```python
from build123d import *

# Parameters (mm, degrees)
SKETCH_1_W                   = 50
SKETCH_1_H                   = 95
EXTRUDE_1_DEPTH              = 20
HOLE_WIZARD_1_D              = 6.4
HOLE_WIZARD_1_CBORE_D        = 11
HOLE_WIZARD_1_CBORE_DEPTH    = 7
HOLE_WIZARD_M4_1_D           = 3.3
HOLE_WIZARD_M4_1_CSINK_D     = 4.05
HOLE_WIZARD_M4_1_CSINK_ANGLE = 90
CHAMFER_1_SIZE               = 1


with BuildPart() as part:
    # 草图1 → 凸台-拉伸1 (new body)
    with BuildSketch(Plane.XY):
        Rectangle(SKETCH_1_W, SKETCH_1_H)
    extrude(amount=EXTRUDE_1_DEPTH)

    # 打孔尺寸(%根据)内六角圆柱头螺钉的类型1 (through all)
    with Locations(Plane(origin=(0, 0, 0), x_dir=(-1, 0, 0), z_dir=(0, 0, -1))):
        with Locations((-19, 30), (-19, -30), (19, -30), (19, 30)):
            CounterBoreHole(HOLE_WIZARD_1_D / 2, HOLE_WIZARD_1_CBORE_D / 2, HOLE_WIZARD_1_CBORE_DEPTH)

    # M4 螺纹孔1 (through all)
    with Locations(Plane(origin=(0, 0, 0), x_dir=(-1, 0, 0), z_dir=(0, 0, -1))):
        with Locations((0, -39), (10, 39), (10, -39), (-10, -39), (-10, 39), (0, 39)):
            CounterSinkHole(HOLE_WIZARD_M4_1_D / 2, HOLE_WIZARD_M4_1_CSINK_D / 2, counter_sink_angle=HOLE_WIZARD_M4_1_CSINK_ANGLE)

    # 倒角1
    chamfer_1_edges = [part.edges().sort_by_distance(p)[0] for p in [
        (25, -47.5, 10),
        (-25, -47.5, 10),
        (-25, 47.5, 10),
        (25, 47.5, 10),
    ]]
    chamfer(chamfer_1_edges, length=CHAMFER_1_SIZE)


solid = part.part
```
For this review, take the finished solid that the model builds, in its own axes (mm). A direction names the side the tool comes from. Round coordinates to 2 decimals unless told otherwise and drop trailing zeros. Write each loop counter-clockwise with the first axis right and the second up, starting at its lowest first coordinate (ties: lowest second). Pieces come first, ordered by that corner, then holes. Notation, with made-up numbers: (60, 48.25) - (79, 48.25) arc R20 ccw to (79, 86.25) - close; hole circle Ø1 at (87.5, -11). An arc over 180 degrees is marked (long way). Answer as a JSON object with one key per item and string values.
1. We need section A-A on z = 13.5. Count the separate pieces of the cut face and the enclosed holes in it, then the cut area to 3 significant figures.
Response values:
{"separate pieces": "1", "enclosed holes": "10", "area": "4,570 mm2"}
2. Tool access review of faces 1 (the face through (10.89, -37.61, 10.32)), 2 (the face through (16.6, -32.4, 7)): name each direction out of +Z, -Z, +X, -X, +Y, -Y from which nothing blocks a thin tool from reaching the whole face with its end or side.
Response values:
{"face 1": "+Z, -Z", "face 2": "-Z"}
3. Draft analysis for pull direction Y (two halves, no side actions). For faces 3 (the face through (-18.284, 35.453, 3.451)), 4 (the face through (0, 47.5, 10)), 5 (the face through (-25, -1, 10)), state which applies: +Y half, -Y half, draft (parallel to the pull), parting line (faces both ways), or undercut.
Response values:
{"face 3": "undercut", "face 4": "+Y half", "face 5": "draft"}
4. For pin 1 Ø10 at (x, y) = (19, 30) entering from -Z, flat-tipped, find the tip position at first contact; note if it passes through.
Response values:
{"pin 1": "stops at z = 7"}
5. We need section B-B on y = -39. Give the boundary of the cut face in (x, z) (3 decimals), then the cut area to 3 significant figures.
Response values:
{"outline": "(-25, 0) - (-12.025, 0) - (-11.65, 0.375) - (-11.65, 20) - (-25, 20) - close; (-8.35, 0.375) - (-7.975, 0) - (-2.025, 0) - (-1.65, 0.375) - (-1.65, 20) - (-8.35, 20) - close; (1.65, 0.375) - (2.025, 0) - (7.975, 0) - (8.35, 0.375) - (8.35, 20) - (1.65, 20) - close; (11.65, 0.375) - (12.025, 0) - (25, 0) - (25, 20) - (11.65, 20) - close", "area": "802 mm2"}
6. We need section C-C on x = -19. Give the boundary of the cut face in (y, z).
Response values:
{"outline": "(-47.5, 0) - (-35.5, 0) - (-35.5, 7) - (-33.2, 7) - (-33.2, 20) - (-47.5, 20) - close; (-26.8, 7) - (-24.5, 7) - (-24.5, 0) - (24.5, 0) - (24.5, 7) - (26.8, 7) - (26.8, 20) - (-26.8, 20) - close; (33.2, 7) - (35.5, 7) - (35.5, 0) - (47.5, 0) - (47.5, 20) - (33.2, 20) - close"}
7. We need section D-D on y = 30. Give the boundary of the cut face in (x, z).
Response values:
{"outline": "(-25, 0) - (-24.5, 0) - (-24.5, 7) - (-22.2, 7) - (-22.2, 20) - (-25, 20) - close; (-15.8, 7) - (-13.5, 7) - (-13.5, 0) - (13.5, 0) - (13.5, 7) - (15.8, 7) - (15.8, 20) - (-15.8, 20) - close; (22.2, 7) - (24.5, 7) - (24.5, 0) - (25, 0) - (25, 20) - (22.2, 20) - close"}
8. To check wall thickness, follow line 1 along Y through (x, z) = (-10, 14); line 2 along Y through (x, z) = (-19, 13); line 3 along X through (y, z) = (39, 5.5). State the ranges of each line that lie inside material, in increasing order.
Response values:
{"line 1": "y = -47.5 to -40.65, -37.35 to 37.35, 40.65 to 47.5", "line 2": "y = -47.5 to -33.2, -26.8 to 26.8, 33.2 to 47.5", "line 3": "x = -25 to -11.65, -8.35 to -1.65, 1.65 to 8.35, 11.65 to 25"}
